Check sheet for the drawn part. Datum: minimum x, y, z corner. Units: mm. Give positions to 0.01 mm unless a question says otherwise; leave off trailing zeros. Loops run counter-clockwise (first coordinate to the right, second up) from the corner with the lowest first, then second, coordinate; pieces in that order, holes last. Notation, with made-up numbers: M 60.25,68.25 L 92.25,68.25 A21 cw 92.25,101.25 Z; hole C 78.25,62 d6. An arc over 180 degrees is marked long. Write each question's results on one line, items separated by ' | '. Start each with the question number.
1. Sectioned sample at B-B on y = 66. Record the cut outline in (x, z).
2. Material ranges on line 1 along Y through (x, z) = (42, 3); line 2 along X through (y, z) = (29.5, 7.75); line 3 along X through (y, z) = (54, 1.5), recorded low to high.
3. Go/stop test with a flat-tipped pin: pin 1 (2 mm diameter, centred on x = 63.5, z = 1.5, fed in from -Y). Record where the tip stops, or that it passes through.
4. Sectioned sample at C-C on x = 64. Record the cut outline in (y, z).
5. Sectioned sample at A-A on z = 13.5. Record the cut outline in (x, y), and give its area (3 significant figures).
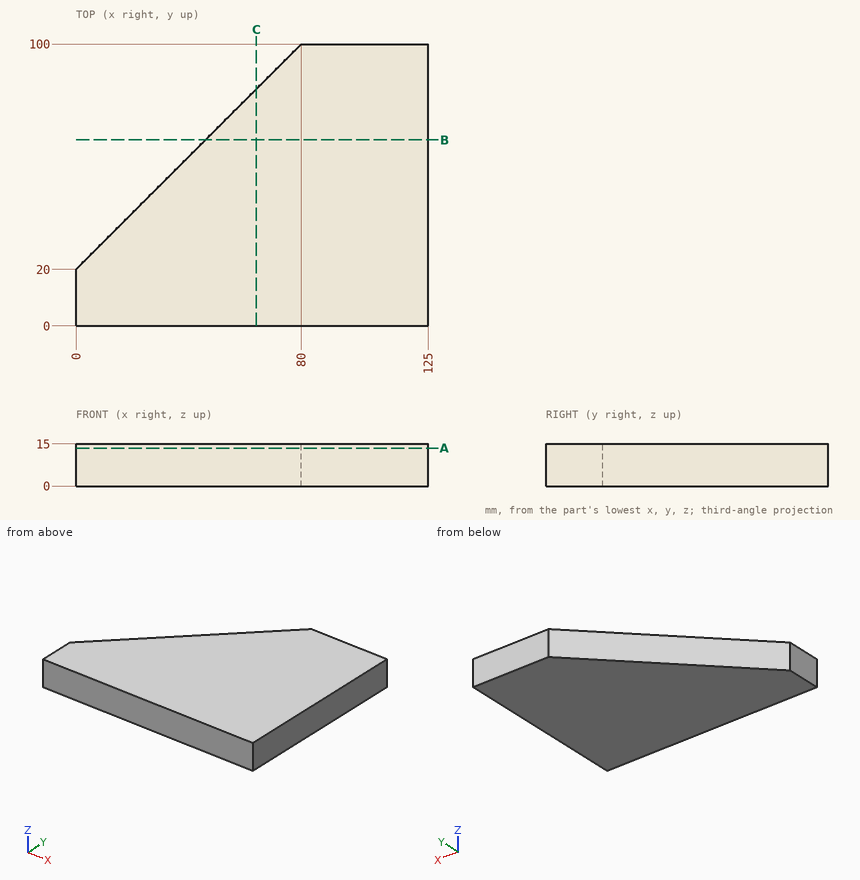
Output values:
1) outline: M 46,0 L 125,0 L 125,15 L 46,15 Z
2) line 1: 0 to 62 | line 2: 9.5 to 125 | line 3: 34 to 125
3) pin 1: y = 0
4) outline: M 0,0 L 84,0 L 84,15 L 0,15 Z
5) outline: M 0,0 L 125,0 L 125,100 L 80,100 L 0,20 Z | area: 9,300 mm2
